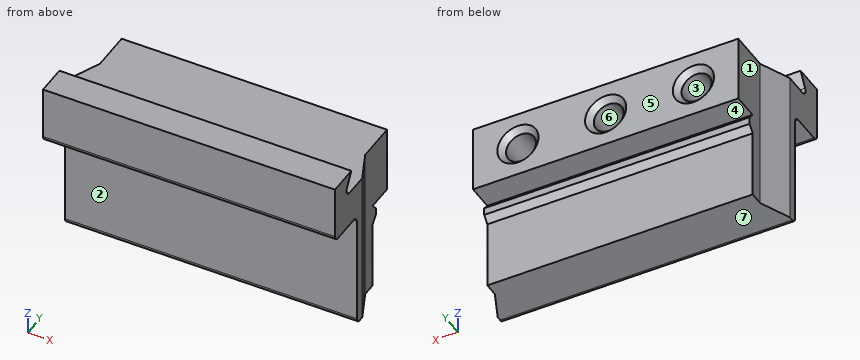
from build123d import *

# Parameters (mm, degrees)
DOVETAIL_BODY_DEPTH       = 48
GROOVE_CUT_DEPTH          = 88
MOUNTING_HOLES_LAYOUT_R   = 4
MOUNTING_HOLES_3X_8_DEPTH = 10
HOLE_CHAMFERS_1_5X45_SIZE = 1.5


with BuildPart() as part:
    # Dovetail Body Profile → Dovetail Body (new body)
    with BuildSketch(Plane.XY):
        Polygon((0, 0), (0, 13.33), (3.561829482, 21.33), (3.561829482, 32), (74.438170518, 32), (74.438170518, 21.33), (78, 13.33), (78, 0), align=None)
    extrude(amount=-DOVETAIL_BODY_DEPTH)

    # Groove Profile → Groove Cut (cut)
    with BuildSketch(Plane(origin=(78, 0, 0), x_dir=(0, 0, -1), z_dir=(1, 0, 0))):
        with BuildLine():
            Line((0, 8), (3.75, 5.834936491))
            ThreePointArc((3.75, 5.834936491), (5.25, 5.834936491), (6, 7.133974596))
            Line((6, 7.133974596), (6, 32))
            Line((6, 32), (0, 32))
            Line((0, 32), (0, 8))
        make_face()
        Polygon((48, 25), (48, 32), (24, 32), (24, 25), (25.787630389, 26.5), (27.787630389, 26.5), (29.575260778, 25), align=None)
        with BuildLine():
            Line((46.5, 10.67), (17.171381992, 10.67))
            ThreePointArc((17.171381992, 10.67), (16.11072182, 10.230660172), (15.671381992, 9.17))
            Line((15.671381992, 9.17), (15.671381992, 1.5))
            ThreePointArc((15.671381992, 1.5), (15.232042164, 0.439339828), (14.171381992, 0))
            Line((14.171381992, 0), (48, 0))
            Line((48, 0), (48, 12.17))
            ThreePointArc((48, 12.17), (47.560660172, 11.109339828), (46.5, 10.67))
        make_face()
    extrude(amount=-GROOVE_CUT_DEPTH, mode=Mode.SUBTRACT)

    # Mounting Holes Layout → Mounting Holes 3xØ8 (cut)
    with BuildSketch(Plane(origin=(0, 32, 0), x_dir=(1, 0, 0), z_dir=(0, 1, 0))):
        with Locations(Location((62.438170518, 15, 0), (0, 0, 270))):
            Circle(MOUNTING_HOLES_LAYOUT_R)
        with Locations(Location((39, 15, 0), (0, 0, 270))):
            Circle(MOUNTING_HOLES_LAYOUT_R)
        with Locations(Location((15.561829482, 15, 0), (0, 0, 270))):
            Circle(MOUNTING_HOLES_LAYOUT_R)
    extrude(amount=-MOUNTING_HOLES_3X_8_DEPTH, mode=Mode.SUBTRACT)

    # Hole Chamfers 1.5x45
    hole_chamfers_1_5x45_edges = [part.edges().sort_by_distance(p)[0] for p in [
        (62.438170518, 32, -19),
        (39, 32, -19),
        (15.561829482, 32, -19),
    ]]
    chamfer(hole_chamfers_1_5x45_edges, length=HOLE_CHAMFERS_1_5X45_SIZE)


solid = part.part
Source: CAD feature listing. Evaluate the final solid. Frame: model axes, mm. Face numbers are marked on the shaded views. A direction names the side the tool comes from. Give positions to 0.01 mm unless a question says otherwise; leave off trailing zeros. Write each loop counter-clockwise with the first axis right and the second up, starting at its lowest first coordinate (ties: lowest second). Pieces come first, ordered by that corner, then holes. Notation, with made-up numbers: M -35.75,5 L 10.25,5 A9 ccw 10.25,10 Z; hole C -39.5,-25 d1. An arc over 180 degrees is marked long. Return JSON: item names as keys, results as strings. Group by question number.
1) Ray query, L1, parallel to X at y = 24, z = -15; L2, parallel to Z at x = 15.5, y = 24.5; L3, parallel to Y at x = 4, z = -32.5. Return the intervals inside material, ascending.
2) Set-up query: the marked faces 1, 2, 3 and 4. Return all of +Z, -Z, +X, -X, +Y, -Y with unobstructed straight access to the full face (end or side cutting, diameter ignored); none if empty.
3) First-contact query: pin 1 Ø5 at (x, z) = (47, -32) entering from -Y; pin 2 Ø12 at (x, z) = (31, -43) entering from +Y; pin 3 Ø1 at (x, y) = (31.5, 13.5) entering from +Z. Flat tips, straight axial feed; report the tip coordinate or a pass-through.
4) Draft query along Z for the marked faces 5, 6 and 7. Return one class per face: released by +Z, released by -Z, zero draft, split by the parting line, or undercut.
5) Cut plane A-A, the plane x = 39. Output: boundary loops of the cut face in (y, z), then the cut area to 3 significant figures.
Data:
{
 "1": {"L1": "x = 3.56 to 11.56, 19.56 to 35, 43 to 58.44, 66.44 to 74.44", "L2": "z = -48 to -19, -11 to -6", "L3": "y = 10.67 to 25"},
 "2": {"face 1": "+Z, -Z, -X, +Y", "face 2": "-Z, +X, -X, -Y", "face 3": "+Y", "face 4": "+X, -X, +Y"},
 "3": {"pin 1": "stops at y = 10.67", "pin 2": "stops at y = 25", "pin 3": "stops at z = -6"},
 "4": {"face 5": "zero draft", "face 6": "undercut", "face 7": "released by -Z"},
 "5": {"outline": "M 0,-14.17 A1.5 ccw 1.5,-15.67 L 9.17,-15.67 A1.5 cw 10.67,-17.17 L 10.67,-46.5 A1.5 ccw 12.17,-48 L 25,-48 L 25,-29.58 L 26.5,-27.79 L 26.5,-25.79 L 25,-24 L 32,-24 L 32,-20.5 L 30.5,-19 L 22,-19 L 22,-11 L 30.5,-11 L 32,-9.5 L 32,-6 L 7.13,-6 A1.5 cw 5.83,-3.75 L 8,0 L 0,0 Z", "area": "793 mm²"}
}
